The listing builds one solid part. Answer for the finished solid, in the listing's coordinates (mm). A direction names the side the tool comes from. Round coordinates to 2 decimals unless told otherwise and drop trailing zeros. Write each loop counter-clockwise with the first axis right and the second up, starting at its lowest first coordinate (ties: lowest second). Pieces come first, ordered by that corner, then holes.
from build123d import *

# Parameters (mm, degrees)
CUT_CIRCLE_75_SKETCH_R        = 37.5
CUT_75_DEPTH                  = 85.113019206
MOUNTING_START                = -28
MOUNTING_FLANGE_SKETCH_R      = 7.5
MOUNTING_FLANGE_3_HOLES_DEPTH = 7.5
HUB_CUT_SKETCH_R              = 37.5
HUB_CUT_DEPTH                 = 139.879868922
HUB_FILLET_R5_R               = 5


with BuildPart() as part:
    # Spigot Profile Sketch → Spigot Body (revolve)
    with BuildSketch(Plane.XY, mode=Mode.PRIVATE) as spigot_body_sk:
        Polygon((0, -13.004960987), (0, 41.995039013), (-45, 41.995039013), (-45, 26.995039013), (-42, 26.995039013), (-42, 16.995039013), (-45, 16.995039013), (-45, -3.004960987), (-42, -3.004960987), (-42, -13.004960987), align=None)
    revolve(spigot_body_sk.sketch.rotate(Axis((0, 45.605381166, 0), (0, -1, 0)), 270), axis=Axis((0, 45.605381166, 0), (0, -1, 0)))

    # Cut Circle Ø75 Sketch → Cut Ø75 (cut, through all)
    with BuildSketch(Plane(origin=(0, 41.995039013, 0), x_dir=(1, 0, 0), z_dir=(0, 1, 0))):
        with Locations(Location((0, 0, 0), (0, 0, 270))):
            Circle(CUT_CIRCLE_75_SKETCH_R)
    extrude(amount=-CUT_75_DEPTH, mode=Mode.SUBTRACT)



with BuildPart() as body_2:
    # Mounting Flange Sketch → Mounting Flange 3 Holes (new body)
    with BuildSketch(Plane(origin=(0, 0, 0), x_dir=(1, 0, 0), z_dir=(0, 1, 0)).offset(MOUNTING_START)):
        with BuildLine():
            ThreePointArc((14.813512184, 76.09647474), (0, 86.05), (-14.813512184, 76.09647474))
            ThreePointArc((-14.813512184, 76.09647474), (-19.247651964, 69.453295695), (-25.927758901, 65.074986119))
            ThreePointArc((-25.927758901, 65.074986119), (-60.665079535, 35.025), (-69.32047058, -10.083395188))
            ThreePointArc((-69.32047058, -10.083395188), (-69.77214443, -18.057692283), (-73.308236355, -25.2193595))
            ThreePointArc((-73.308236355, -25.2193595), (-74.521485996, -43.025), (-58.494724172, -50.87711524))
            ThreePointArc((-58.494724172, -50.87711524), (-50.524492466, -51.395603412), (-43.392711679, -54.991590931))
            ThreePointArc((-43.392711679, -54.991590931), (0, -70.05), (43.392711679, -54.991590931))
            ThreePointArc((43.392711679, -54.991590931), (50.524492466, -51.395603412), (58.494724172, -50.87711524))
            ThreePointArc((58.494724172, -50.87711524), (74.521485996, -43.025), (73.308236355, -25.2193595))
            ThreePointArc((73.308236355, -25.2193595), (69.77214443, -18.057692283), (69.32047058, -10.083395188))
            ThreePointArc((69.32047058, -10.083395188), (60.665079535, 35.025), (25.927758901, 65.074986119))
            ThreePointArc((25.927758901, 65.074986119), (19.247651964, 69.453295695), (14.813512184, 76.09647474))
        make_face()
        with Locations(Location((0, 70.05, 0), (0, 0, 270))):
            Circle(MOUNTING_FLANGE_SKETCH_R, mode=Mode.SUBTRACT)
        with Locations(Location((60.665079535, -35.025, 0), (0, 0, 270))):
            Circle(MOUNTING_FLANGE_SKETCH_R, mode=Mode.SUBTRACT)
        with Locations(Location((-60.665079535, -35.025, 0), (0, 0, 270))):
            Circle(MOUNTING_FLANGE_SKETCH_R, mode=Mode.SUBTRACT)
    extrude(amount=-MOUNTING_FLANGE_3_HOLES_DEPTH)


with BuildPart() as part_1:
    add(part.part)

    add(body_2.part)  # Flange Hub merges body 2
    # Flange Hub Profile Sketch → Flange Hub (revolve)
    with BuildSketch(Plane.XY, mode=Mode.PRIVATE) as flange_hub_sk:
        Polygon((-45, -28), (0, -28), (0, -13.004960987), (-42, -13.004960987), (-45, -13.004960987), (-45, -23), align=None)
    revolve(flange_hub_sk.sketch.rotate(Axis((0, 0, 0), (0, -1, 0)), 270), axis=Axis((0, 0, 0), (0, -1, 0)))

    # Hub Cut Sketch → Hub Cut (cut, through all)
    with BuildSketch(Plane(origin=(0, 41.995039013, 0), x_dir=(1, 0, 0), z_dir=(0, 1, 0))):
        with Locations(Location((0, 0, 0), (0, 0, 270))):
            Circle(HUB_CUT_SKETCH_R)
    extrude(amount=-HUB_CUT_DEPTH, mode=Mode.SUBTRACT)

    # Hub Fillet R5
    hub_fillet_r5_edges = [part_1.edges().sort_by_distance(p)[0] for p in [
        (0, -28, -45),
    ]]
    fillet(hub_fillet_r5_edges, radius=HUB_FILLET_R5_R)


solid = part_1.part
1. Section A-A on x = 0 is taken. Give the number of separate pieces and of enclosed holes in the cut face, plus the area to 3 significant figures.
Geometry says:
separate pieces: 3
enclosed holes: 0
area: 1,440 mm2
2. Section D-D on z = -70.05 is taken. Determine the outline of the cut face in (x, y), plus the area to 3 significant figures.
Geometry says:
outline: (-18.67, -35.5) - (-7.5, -35.5) - (-7.5, -28) - (-18.67, -28) - close; (7.5, -35.5) - (18.67, -35.5) - (18.67, -28) - (7.5, -28) - close
area: 168 mm2
3. For a pull along X with two mould halves and no side action, classify faces 4 (the face through (-69.744, -31.697, 17.949)), 5 (the face through (50.416, -31.697, 51.426)), 6 (the face through (-0.655, -31.697, 70.047)), 7 (the face through (-22.818, 3.79, -29.759)) as released by +X, released by -X, zero draft, split by the parting line, or undercut.
Geometry says:
face 4: released by -X
face 5: undercut
face 6: split by the parting line
face 7: undercut
4. Section C-C on y = 8 is taken. Determine the outline of the cut face in (x, z).
Geometry says:
outline: circle Ø90 at (0, 0); hole circle Ø75 at (0, 0)
5. Straight lines are drawn through the part: line 1 along X through (y, z) = (37.5, -1); line 2 along X through (y, z) = (34, -19.5); line 3 along Z through (x, y) = (10, -29). For each, find the intervals that lie inside material, in ascending order.
Geometry says:
line 1: x = -44.99 to -37.49, 37.49 to 44.99
line 2: x = -40.56 to -32.03, 32.03 to 40.56
line 3: z = -82.54 to -36.14, 36.14 to 69.33
6. A tool of negligible diameter and unlimited length cuts with its end or side. For faces 1 (the face through (0.265, -31.697, -86.048)), 2 (the face through (50, -28, 8)), 3 (the face through (40, 16.995, 14)), from which of +Z, -Z, +X, -X, +Y, -Y can it reach the whole face along a straight path? Write none if from no direction.
Geometry says:
face 1: -Z, +Y, -Y
face 2: +Y
face 3: none
7. Given pin 1 (2 mm diameter, centred on x = -45.5, y = 25.5, fed in from -Z); pin 2 (8 mm diameter, centred on y = -18.5, z = 26.5, fed in from -X); pin 3 (19.5 mm diameter, centred on x = 0, z = -70.05, fed in from +Y); pin 4 (10 mm diameter, centred on x = 31, y = -2.5, fed in from -Z), each flat-ended and moving along its own axis, determine where each tip first touches the part or whether it passes through.
Geometry says:
pin 1: passes through
pin 2: stops at x = -38.97
pin 3: stops at y = -28
pin 4: stops at z = -36.73
